```python
from build123d import *

# Parameters (mm, degrees)
BOSS_EXTRUDE1_DEPTH        = 8
F_12_0_12_DIAMETER_HOLE1_D = 12


with BuildPart() as part:
    # Sketch1 → Boss-Extrude1 (new body)
    with BuildSketch(Plane.XY):
        with BuildLine():
            Line((-1275, 69.282032303), (-1235, 0))
            ThreePointArc((-1235, 0), (0, 330.917252652), (1235, 0))
            Line((1235, 0), (1275, 69.282032303))
            ThreePointArc((1275, 69.282032303), (0, 410.917252652), (-1275, 69.282032303))
        make_face()
    extrude(amount=BOSS_EXTRUDE1_DEPTH)

    # Ø12.0 (12) Diameter Hole1 (through all)
    with Locations(Plane.XY.offset(8)):
        with Locations((-1227.328979234, 76.713402287), (-1207.947550426, 41.722543232), (248.497397062, 381.698489423), (244.573237614, 341.891442652), (337.892259182, 371.279342309), (332.556416163, 331.636830036)):
            Hole(F_12_0_12_DIAMETER_HOLE1_D / 2)


solid = part.part
```
Verification items for the finished model (mm, model axes). Coordinates: 2 decimals unless noted, no trailing zeros. Write each loop counter-clockwise with the first axis right and the second up, starting at its lowest first coordinate (ties: lowest second). Pieces come first, ordered by that corner, then holes. Notation, with made-up numbers: M -28,1 L 30,1 A31 ccw 30,40 Z; hole C 11,52 d3. An arc over 180 degrees is marked long. Answer as a JSON object with one key per item and string values. Group by question number.
(1) Cross-section at B-B, the plane z = 4.5. Record the cut outline in (x, y).
(2) Gauge pin test, flat ends, axial feed: pin 1 (1 mm diameter, centred on y = 161.5, z = 3.5, fed in from -X); pin 2 (4 mm diameter, centred on x = -790.5, z = 3.5, fed in from +Y). Record the tip position at first contact, or that the pin passes through.
(3) Material ranges on line 1 (X direction, y = 68, z = 6.5); line 2 (Y direction, x = 8, z = 2); line 3 (X direction, y = 84.5, z = 5.5), recorded low to high.
(4) Cross-section at A-A, the plane y = 261. Record the cut outline in (x, z).
(5) Release check for a two-part mould opening along X. For faces 1 (the face through (18.69, 410.85, 3.94)), 2 (the face through (-18.11, 330.85, 3.94)), 3 (the face through (-1255.28, 35.126, 3.944)) record: +X half, -X half, draft (parallel to the pull), parting line (faces both ways), or undercut.
(6) Cross-section at C-C, the plane y = 165.5. Record the cut outline in (x, z).
(7) Cross-section at D-D, the plane x = -283. Record the cut outline in (y, z).
Reply:
{
 "1": {"outline": "M -1275,69.28 L -1235,0 A2470 cw 1235,0 L 1275,69.28 A2550 ccw Z; hole C -1227.33,76.71 d12; hole C -1207.95,41.72 d12; hole C 244.57,341.89 d12; hole C 248.5,381.7 d12; hole C 332.56,331.64 d12; hole C 337.89,371.28 d12"},
 "2": {"pin 1": "x = -1100.96", "pin 2": "y = 285.95"},
 "3": {"line 1": "-1274.26 to -1108.91, 1108.91 to 1274.26", "line 2": "330.9 to 410.9", "line 3": "-1248.27 to -1075.44, 1075.44 to 1248.27"},
 "4": {"outline": "M -861.45,0 L -583.53,0 L -583.53,8 L -861.45,8 Z; M 583.53,0 L 861.45,0 L 861.45,8 L 583.53,8 Z"},
 "5": {"face 1": "parting line", "face 2": "undercut", "face 3": "-X half"},
 "6": {"outline": "M -1091.51,0 L -888.71,0 L -888.71,8 L -1091.51,8 Z; M 888.71,0 L 1091.51,0 L 1091.51,8 L 888.71,8 Z"},
 "7": {"outline": "M 314.65,0 L 395.16,0 L 395.16,8 L 314.65,8 Z"}
}
